from build123d import *

# Parameters (mm, degrees)
GB_6728_1986_050_X_50_X_3_1_DEPTH = 800


with BuildPart() as part:
    # Sketch1 → Gb／6728-1986方形空心型钢 050 X 50 X 3(1) (new body)
    with BuildSketch(Plane.YX.offset(-400)):
        with BuildLine():
            Line((-19, -25), (19, -25))
            ThreePointArc((19, -25), (23.242640687, -23.242640687), (25, -19))
            Line((25, -19), (25, 19))
            ThreePointArc((25, 19), (23.242640687, 23.242640687), (19, 25))
            Line((19, 25), (-19, 25))
            ThreePointArc((-19, 25), (-23.242640687, 23.242640687), (-25, 19))
            Line((-25, 19), (-25, -19))
            ThreePointArc((-25, -19), (-23.242640687, -23.242640687), (-19, -25))
        make_face()
        with BuildLine():
            Line((-19, -22), (19, -22))
            ThreePointArc((19, -22), (21.121320344, -21.121320344), (22, -19))
            Line((22, -19), (22, 19))
            ThreePointArc((22, 19), (21.121320344, 21.121320344), (19, 22))
            Line((19, 22), (-19, 22))
            ThreePointArc((-19, 22), (-21.121320344, 21.121320344), (-22, 19))
            Line((-22, 19), (-22, -19))
            ThreePointArc((-22, -19), (-21.121320344, -21.121320344), (-19, -22))
        make_face(mode=Mode.SUBTRACT)
    extrude(amount=GB_6728_1986_050_X_50_X_3_1_DEPTH)


solid = part.part
Read the model definition and answer for the solid it produces. Units are mm, in the model's axes. A direction names the side the tool comes from. Give positions to 0.01 mm unless a question says otherwise; leave off trailing zeros. Loops run counter-clockwise (first coordinate to the right, second up) from the corner with the lowest first, then second, coordinate; pieces in that order, holes last. Notation, with made-up numbers: (45.5, 69.25) -> (60.5, 69.25) arc R20 ccw to (60.5, 73.25) -> close; hole circle Ø8 at (56, -21). An arc over 180 degrees is marked (long way). Answer as CSV lines item,"result".
Item 1: Find section A-A on x = 4. Give the vertices of the cut face in (y, z), plus the area to 3 significant figures.
Returned:
outline,"(-25, -400) -> (-22, -400) -> (-22, 400) -> (-25, 400) -> close; (22, -400) -> (25, -400) -> (25, 400) -> (22, 400) -> close"
area,"4,800 mm²"
Item 2: Find section C-C on z = 251.5. Give the vertices of the cut face in (x, y).
Returned:
outline,"(-25, -19) arc R6 ccw to (-19, -25) -> (19, -25) arc R6 ccw to (25, -19) -> (25, 19) arc R6 ccw to (19, 25) -> (-19, 25) arc R6 ccw to (-25, 19) -> close; hole (-22, -19) arc R3 ccw to (-19, -22) -> (19, -22) arc R3 ccw to (22, -19) -> (22, 19) arc R3 ccw to (19, 22) -> (-19, 22) arc R3 ccw to (-22, 19) -> close"
Item 3: For faces 5 (the face through (25, 0, 6)), 6 (the face through (22, 0, 6)), determine the directions among +Z, -Z, +X, -X, +Y, -Y from which every point of the face is accessible in a straight line to the end or side of a thin tool.
Returned:
face 5,"+Z, -Z, +X, +Y, -Y"
face 6,"+Z, -Z"
Item 4: Determine the mould class of faces 1 (the face through (-25, 0, 6)), 2 (the face through (0.1, -22.3, -400)), 3 (the face through (-22, 0, 6)), 4 (the face through (0, 22, 6)) for opening direction X: +X half, -X half, draft (parallel to the pull), parting line (faces both ways), or undercut.
Returned:
face 1,"-X half"
face 2,"draft"
face 3,"undercut"
face 4,"undercut"
Item 5: Consider line 1 (Y direction, x = 14.5, z = 249); line 2 (Y direction, x = -21, z = -265.5). Determine where each line is inside the solid, lowest interval first. Write a range as [from, to].
Returned:
line 1,"y = [-25, -22], [22, 25]"
line 2,"y = [-24.66, -21.24], [21.24, 24.66]"
